The model under review builds one solid part; all positions refer to its coordinate system, in mm. A direction names the side the tool comes from. Round coordinates to 2 decimals unless told otherwise and drop trailing zeros. Write each loop counter-clockwise with the first axis right and the second up, starting at its lowest first coordinate (ties: lowest second). Pieces come first, ordered by that corner, then holes. Notation, with made-up numbers: (-8.5, 65) - (41.5, 65) arc R15 ccw to (41.5, 88) - close; hole circle Ø5 at (5.25, 40.25). An arc over 180 degrees is marked (long way). Return JSON: item names as keys, results as strings.
from build123d import *

# Parameters (mm, degrees)
SKETCH_1_W                = 25
SKETCH_1_H                = 40
EXTRUDE_1_DEPTH           = 5
CUT_EXTRUDE_1_DEPTH       = 10
CHAMFER_1_SIZE            = 1
HOLE_WIZARD_1_D           = 4.5
HOLE_WIZARD_1_CBORE_D     = 8
HOLE_WIZARD_1_CBORE_DEPTH = 4.6
HOLE_WIZARD_M4_1_D        = 4.5


with BuildPart() as part:
    # 草图1 → 凸台-拉伸1 (new, symmetric)
    with BuildSketch(Plane(origin=(0, 0, 0), x_dir=(1, 0, 0), z_dir=(0, 1, 0))):
        Rectangle(SKETCH_1_W, SKETCH_1_H)
    extrude(amount=EXTRUDE_1_DEPTH, both=True)

    # 草图2 → 切除-拉伸1 (cut)
    with BuildSketch(Plane(origin=(0, 5, 0), x_dir=(1, 0, 0), z_dir=(0, 1, 0))):
        with BuildLine():
            Line((12.5, -20), (-2.5, -20))
            Line((-2.5, -20), (-2.5, 7))
            ThreePointArc((-2.5, 7), (-1.621320344, 9.121320344), (0.5, 10))
            Line((0.5, 10), (12.5, 10))
            Line((12.5, 10), (12.5, -20))
        make_face()
    extrude(amount=-CUT_EXTRUDE_1_DEPTH, mode=Mode.SUBTRACT)

    # 倒角1
    chamfer_1_edges = [part.edges().sort_by_distance(p)[0] for p in [
        (-2.5, 0, 20),
        (12.5, 0, -10),
    ]]
    chamfer(chamfer_1_edges, length=CHAMFER_1_SIZE)

    # 打孔尺寸(%根据)内六角圆柱头螺钉的类型1 (through all)
    with Locations(Plane(origin=(-2.5, 0, 0), x_dir=(0, 0, -1), z_dir=(1, 0, 0))):
        with Locations((-15, 0), (0, 0)):
            CounterBoreHole(HOLE_WIZARD_1_D / 2, HOLE_WIZARD_1_CBORE_D / 2, HOLE_WIZARD_1_CBORE_DEPTH)

    # M4 间隙孔1 (through all)
    with Locations(Plane.XY.offset(-10)):
        with Locations((7.5, 0)):
            Hole(HOLE_WIZARD_M4_1_D / 2)


solid = part.part
(1) Clearance check with flat-ended pins moving along their axes: pin 1 Ø1 at (x, y) = (8.5, -3.5) entering from +Z; pin 2 Ø2.5 at (y, z) = (-0.5, -1) entering from +X. State where each tip first meets the part, or that it passes through.
Filled in:
{"pin 1": "stops at z = -10", "pin 2": "stops at x = -7.1"}
(2) Add section A-A (z = 0). Write out the cut boundary in (x, y).
Filled in:
{"outline": "(-12.5, -5) - (-2.5, -5) - (-2.5, -4) - (-7.1, -4) - (-7.1, -2.25) - (-12.5, -2.25) - close; (-12.5, 2.25) - (-7.1, 2.25) - (-7.1, 4) - (-2.5, 4) - (-2.5, 5) - (-12.5, 5) - close"}
(3) Add section C-C (y = 4.5). Write out the cut boundary in (x, z).
Filled in:
{"outline": "(-12.5, -20) - (12.5, -20) - (12.5, -11) - (11.5, -10) - (0.5, -10) arc R3 cw to (-2.5, -7) - (-2.5, 19) - (-3.5, 20) - (-12.5, 20) - close"}
(4) Wall thickness on line 1 (Y direction, x = -10.05, z = 15); line 2 (Z direction, x = -10.5, y = 1.5); line 3 (Z direction, x = -4.5, y = -2.5): over which ranges is each line inside the solid? List them lowest first.
Filled in:
{"line 1": "y = -5 to -2.25, 2.25 to 5", "line 2": "z = -20 to -1.68, 1.68 to 13.32, 16.68 to 20", "line 3": "z = -20 to -3.12, 3.12 to 11.88, 18.12 to 20"}
(5) For faces 1 (the cylindrical face through (-9.84, 2.23, -0.29)), 2 (the cylindrical face through (-5, 0, 19)), 3 (the flat face through (5, 0, -10)), list the 3-axis set-ups (+Z, -Z, +X, -X, +Y, -Y) from which the entire face can be reached by the end or side of a thin tool; tool diameter is ignored.
Filled in:
{"face 1": "+X, -X", "face 2": "+X", "face 3": "+Z, +X, +Y, -Y"}
(6) Add section D-D (z = -13). Write out the cut boundary in (x, y).
Filled in:
{"outline": "(-12.5, -5) - (12.5, -5) - (12.5, 5) - (-12.5, 5) - close; hole circle Ø4.5 at (7.5, 0)"}
(7) Add section B-B (x = 7.5). Write out the cut boundary in (y, z), plus the area to 3 significant figures.
Filled in:
{"outline": "(-5, -20) - (-2.25, -20) - (-2.25, -10) - (-5, -10) - close; (2.25, -20) - (5, -20) - (5, -10) - (2.25, -10) - close", "area": "55.0 mm2"}
(8) Mouldability with a two-part tool opening along Z and no side actions: class faces 4 (the cylindrical face through (-4.768, -3.905, 0.867)), 5 (the flat face through (-2.5, 0, 6)), 6 (the flat face through (12, 0.1, -10.5)), 7 (the cylindrical face through (-9.838, 0.676, 17.146)) as released by +Z, released by -Z, zero draft, split by the parting line, or undercut.
Filled in:
{"face 4": "undercut", "face 5": "zero draft", "face 6": "released by +Z", "face 7": "undercut"}
